The listing builds one solid part. Answer for the finished solid, in the listing's coordinates (mm). A direction names the side the tool comes from. Coordinates: 2 decimals unless noted, no trailing zeros. Loops run counter-clockwise (first coordinate to the right, second up) from the corner with the lowest first, then second, coordinate; pieces in that order, holes last. Notation, with made-up numbers: (27, -11.75) - (70, -11.75) arc R11 cw to (70, -1.75) - close; hole circle Ø6 at (-31, 65.5). An arc over 180 degrees is marked (long way). Put each result on its own line as item: value.
```python
from build123d import *

# Parameters (mm, degrees)
BOSS_EXTRUDE1_DEPTH = 40
SKETCH2_R           = 1.5
CUT_EXTRUDE1_DEPTH  = 73.972597597


with BuildPart() as part:
    # Sketch1 → Boss-Extrude1 (new body)
    with BuildSketch(Plane.XY):
        Polygon((0, 0), (-25, 0), (-25, 30), (-50, 30), (-50, 35), (-20, 35), (-20, 5), (0, 5), (20, 5), (20, 35), (50, 35), (50, 30), (25, 30), (25, 0), align=None)
    extrude(amount=BOSS_EXTRUDE1_DEPTH)

    # Sketch2 → Cut-Extrude1 (cut, through all)
    with BuildSketch(Plane(origin=(0, 35, 0), x_dir=(1, 0, 0), z_dir=(0, 1, 0))):
        with Locations(Location((-40, -7.5, 0), (0, 0, 180))):
            Circle(SKETCH2_R)
        with Locations(Location((-40, -20, 0), (0, 0, 180))):
            Circle(SKETCH2_R)
        with Locations(Location((-40, -32.5, 0), (0, 0, 180))):
            Circle(SKETCH2_R)
        with Locations(Location((40, -7.5, 0), (0, 0, 180))):
            Circle(SKETCH2_R)
        with Locations(Location((40, -20, 0), (0, 0, 180))):
            Circle(SKETCH2_R)
        with Locations(Location((40, -32.5, 0), (0, 0, 180))):
            Circle(SKETCH2_R)
    extrude(amount=-CUT_EXTRUDE1_DEPTH, mode=Mode.SUBTRACT)


solid = part.part
```
1) Straight lines are drawn through the part: L1, parallel to Z at x = -40, y = 31; L2, parallel to X at y = 18.5, z = 19; L3, parallel to Y at x = 45.5, z = 20.5. For each, find the intervals that lie inside material, in ascending order. Write a range as [from, to].
Found:
L1: z = [0, 6], [9, 18.5], [21.5, 31], [34, 40]
L2: x = [-25, -20], [20, 25]
L3: y = [30, 35]
2) For a pull along Z with two mould halves and no side action, classify faces 5 (the face through (-3.5, 4.6, 40)), 6 (the face through (41.11, 32.53, 21.01)), 7 (the face through (-3.5, 4.6, 0)), 8 (the face through (0, 5, 20)) as pulls with the +Z half, pulls with the -Z half, needs draft (parallel to the pull), parting line crosses it, or undercut.
Found:
face 5: pulls with the +Z half
face 6: undercut
face 7: pulls with the -Z half
face 8: needs draft
3) The part is cut by section D-D (y = 27.5). Give the vertices of the cut face in (x, z), and give its area (3 significant figures).
Found:
outline: (-25, 0) - (-20, 0) - (-20, 40) - (-25, 40) - close; (20, 0) - (25, 0) - (25, 40) - (20, 40) - close
area: 400 mm^2
4) The part is cut by section C-C (y = 31.5). Give the vertices of the cut face in (x, z).
Found:
outline: (-50, 0) - (-20, 0) - (-20, 40) - (-50, 40) - close; (20, 0) - (50, 0) - (50, 40) - (20, 40) - close; hole circle Ø3 at (-40, 7.5); hole circle Ø3 at (-40, 20); hole circle Ø3 at (-40, 32.5); hole circle Ø3 at (40, 7.5); hole circle Ø3 at (40, 20); hole circle Ø3 at (40, 32.5)
5) The part is cut by section B-B (x = -40). Give the vertices of the cut face in (y, z).
Found:
outline: (30, 0) - (35, 0) - (35, 6) - (30, 6) - close; (30, 9) - (35, 9) - (35, 18.5) - (30, 18.5) - close; (30, 21.5) - (35, 21.5) - (35, 31) - (30, 31) - close; (30, 34) - (35, 34) - (35, 40) - (30, 40) - close
6) The part is cut by section A-A (z = 32.5). Give the vertices of the cut face in (x, y), and give its area (3 significant figures).
Found:
outline: (-50, 30) - (-41.5, 30) - (-41.5, 35) - (-50, 35) - close; (-38.5, 30) - (-25, 30) - (-25, 0) - (25, 0) - (25, 30) - (38.5, 30) - (38.5, 35) - (20, 35) - (20, 5) - (-20, 5) - (-20, 35) - (-38.5, 35) - close; (41.5, 30) - (50, 30) - (50, 35) - (41.5, 35) - close
area: 770 mm^2
7) Each of these flat-tipped pins is pushed along its axis until it touches: pin 1 (1.8 mm diameter, centred on x = 40, z = 7.5, fed in from +Y); pin 2 (15 mm diameter, centred on y = 15.5, z = 25, fed in from -X); pin 3 (15 mm diameter, centred on y = 19, z = 21, fed in from +X); pin 4 (12 mm diameter, centred on x = -29.5, y = 21.5, fed in from -Z). Where does it stop, or does it pass through?
Found:
pin 1: passes through
pin 2: stops at x = -25
pin 3: stops at x = 25
pin 4: stops at z = 0
8) For faces 1 (the face through (41.2, 32.5, 31.6)), 2 (the face through (-25, 15, 20)), 3 (the face through (20, 20, 20)), 4 (the face through (25, 15, 20)), determine the directions among +Z, -Z, +X, -X, +Y, -Y from which every point of the face is accessible in a straight line to the end or side of a thin tool.
Found:
face 1: +Y, -Y
face 2: +Z, -Z, -X, -Y
face 3: +Z, -Z, +Y
face 4: +Z, -Z, +X, -Y
